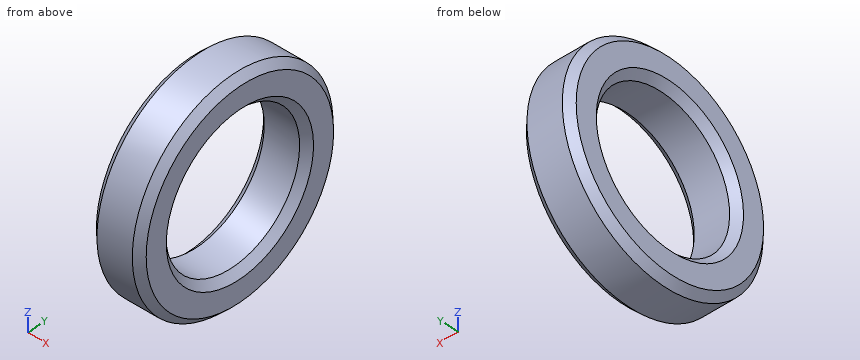
```python
from build123d import *

# Parameters (mm, degrees)
SKETCH1_R           = 15
SKETCH1_R_2         = 10
BOSS_EXTRUDE1_DEPTH = 6.9
CHAMFER1_SIZE       = 1


with BuildPart() as part:
    # Sketch1 → Boss-Extrude1 (new body)
    with BuildSketch(Plane(origin=(0, 0, 0), x_dir=(0, 0, -1), z_dir=(1, 0, 0))):
        with Locations(Location((0, 0, 0), (0, 0, 180))):
            Circle(SKETCH1_R)
        with Locations(Location((0, 0, 0), (0, 0, 180))):
            Circle(SKETCH1_R_2, mode=Mode.SUBTRACT)
    extrude(amount=BOSS_EXTRUDE1_DEPTH)

    # Chamfer1
    chamfer1_edges = [part.edges().sort_by_distance(p)[0] for p in [
        (0, 0, -15),
        (6.9, 0, -15),
        (0, 0, -10),
        (6.9, 0, -10),
    ]]
    chamfer(chamfer1_edges, length=CHAMFER1_SIZE)


solid = part.part
```
The model under review builds one solid part; all positions refer to its coordinate system, in mm. Round coordinates to 2 decimals unless told otherwise and drop trailing zeros. Order: outer loops, then holes, each group sorted by start corner. A loop starts at its lowest first (then second) coordinate and runs counter-clockwise, first axis right, second up. Notation, with made-up numbers: (67.25, 18) -> (124.25, 18) arc R23 cw to (124.25, 33) -> close; hole circle Ø9 at (17.25, -30.75). An arc over 180 degrees is marked (long way). Use a Markdown table: item, result.
Q1. Clearance check with flat-ended pins moving along their axes: P1, Ø2, axis at x = 6, y = 0, coming from the -Z side; P2, Ø1, axis at x = 5.5, z = 6.5, coming from the +Y side; P3, Ø1, axis at x = 2, y = 1, coming from the +Z side; P4, Ø2, axis at x = 1.5, y = -5, coming from the +Z side. State where each tip first meets the part, or that it passes through.
Values:
| item | result |
|---|---|
| P1 | stops at z = -15 |
| P2 | stops at y = 13.75 |
| P3 | stops at z = 14.99 |
| P4 | stops at z = 14.46 |
Q2. For line 1 (Y direction, x = 2.4, z = 0); line 2 (Y direction, x = 1.5, z = -6.25); line 3 (Z direction, x = 3, y = 6.75), list the stretches that pass through material, from the lowest coordinate up.
Values:
| item | result |
|---|---|
| line 1 | y = -15 to -10, 10 to 15 |
| line 2 | y = -13.64 to -7.81, 7.81 to 13.64 |
| line 3 | z = -13.4 to -7.38, 7.38 to 13.4 |
Q3. We need section A-A on y = 0. Write out the cut boundary in (x, z).
Values:
| item | result |
|---|---|
| outline | (0, -14) -> (1, -15) -> (5.9, -15) -> (6.9, -14) -> (6.9, -11) -> (5.9, -10) -> (1, -10) -> (0, -11) -> close; (0, 11) -> (1, 10) -> (5.9, 10) -> (6.9, 11) -> (6.9, 14) -> (5.9, 15) -> (1, 15) -> (0, 14) -> close |
Q4. We need section D-D on x = 4. Write out the cut boundary in (y, z).
Values:
| item | result |
|---|---|
| outline | circle Ø30 at (0, 0); hole circle Ø20 at (0, 0) |
Q5. We need section C-C on x = 6.25. Write out the cut boundary in (y, z), then the cut area to 3 significant figures.
Values:
| item | result |
|---|---|
| outline | circle Ø29.3 at (0, 0); hole circle Ø20.7 at (0, 0) |
| area | 338 mm^2 |
